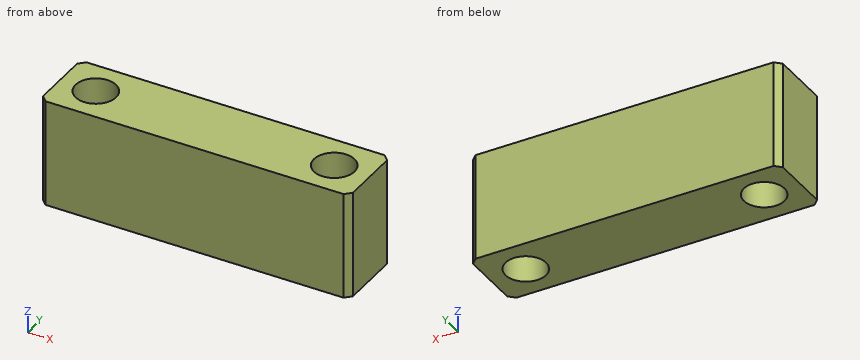
from build123d import *

# Parameters (mm, degrees)
SKETCH1_W                = 26
SKETCH1_H                = 6
BOSS_EXTRUDE1_DEPTH      = 9
M3_CLEARANCE_HOLE1_D     = 3.4
M3_CLEARANCE_HOLE1_DEPTH = 30
M3_CLEARANCE_HOLE1_TIP   = 1.021463052
CHAMFER1_SIZE            = 0.5


with BuildPart() as part:
    # Sketch1 → Boss-Extrude1 (new body)
    with BuildSketch(Plane.XY):
        Rectangle(SKETCH1_W, SKETCH1_H)
    extrude(amount=BOSS_EXTRUDE1_DEPTH)

    # M3 Clearance Hole1
    with Locations(Plane.XY.offset(9)):
        with Locations((-10, 0), (10, 0)):
            Hole(M3_CLEARANCE_HOLE1_D / 2, depth=M3_CLEARANCE_HOLE1_DEPTH)
            with Locations((0, 0, -(M3_CLEARANCE_HOLE1_DEPTH + M3_CLEARANCE_HOLE1_TIP / 2))):  # 118° drill point
                Cone(0, M3_CLEARANCE_HOLE1_D / 2, M3_CLEARANCE_HOLE1_TIP, mode=Mode.SUBTRACT)

    # Chamfer1
    chamfer1_edges = [part.edges().sort_by_distance(p)[0] for p in [
        (13, -3, 4.5),
        (-13, -3, 4.5),
        (-13, 3, 4.5),
        (13, 3, 4.5),
    ]]
    chamfer(chamfer1_edges, length=CHAMFER1_SIZE)


solid = part.part
Check sheet for the modelled part. Datum: model origin and axes. Units: mm. Round coordinates to 2 decimals unless told otherwise and drop trailing zeros. Order: outer loops, then holes, each group sorted by start corner. A loop starts at its lowest first (then second) coordinate and runs counter-clockwise, first axis right, second up.
(1) Go/stop test with a flat-tipped pin: P1, Ø2.5, axis at x = 10, y = 0, coming from the -Z side. Record where the tip stops, or that it passes through.
(2) Cross-section at B-B, the plane x = -10. Enter the section's corners in (y, z), and give its area (3 significant figures).
(3) Scan lines: probe 1 along Y at (x, z) = (10, 7); probe 2 along X at (y, z) = (1.5, 2); probe 3 along X at (y, z) = (-1.1, 0.75). Record each from-to range of solid material in increasing order.
(4) Cross-section at A-A, the plane y = 0. Enter the section's corners in (x, z).
(5) Cross-section at D-D, the plane y = 1.35. Enter the section's corners in (x, z).
(6) Cross-section at C-C, the plane z = 2.5. Enter the section's corners in (x, y), and give its area (3 significant figures).
Check sheet entries:
1. P1: passes through
2. outline: (-3, 0) - (-1.7, 0) - (-1.7, 9) - (-3, 9) - close; (1.7, 0) - (3, 0) - (3, 9) - (1.7, 9) - close
2. area: 23.4 mm2
3. probe 1: y = -3 to -1.7, 1.7 to 3
3. probe 2: x = -13 to -10.8, -9.2 to 9.2, 10.8 to 13
3. probe 3: x = -13 to -11.3, -8.7 to 8.7, 11.3 to 13
4. outline: (-13, 0) - (-11.7, 0) - (-11.7, 9) - (-13, 9) - close; (-8.3, 0) - (8.3, 0) - (8.3, 9) - (-8.3, 9) - close; (11.7, 0) - (13, 0) - (13, 9) - (11.7, 9) - close
5. outline: (-13, 0) - (-11.03, 0) - (-11.03, 9) - (-13, 9) - close; (-8.97, 0) - (8.97, 0) - (8.97, 9) - (-8.97, 9) - close; (11.03, 0) - (13, 0) - (13, 9) - (11.03, 9) - close
6. outline: (-13, -2.5) - (-12.5, -3) - (12.5, -3) - (13, -2.5) - (13, 2.5) - (12.5, 3) - (-12.5, 3) - (-13, 2.5) - close; hole circle Ø3.4 at (-10, 0); hole circle Ø3.4 at (10, 0)
6. area: 137 mm2
